from build123d import *

# Parameters (mm, degrees)
EXTRUDE_1_DEPTH      = 20
EXTRUDE_1_DEPTH_BACK = 10
SKETCH_1_R           = 11.4
SKETCH_2_R           = 12.5
EXTRUDE_2_DEPTH      = 30


with BuildPart() as part:
    # 草图1 → 凸台-拉伸1 (new, two sides: drawn at the far end of the back side and taken through both)
    with BuildSketch(Plane.XY.offset(-EXTRUDE_1_DEPTH_BACK)):
        Circle(SKETCH_1_R)
    extrude(amount=EXTRUDE_1_DEPTH + EXTRUDE_1_DEPTH_BACK)

    # 草图2 → 凸台-拉伸2 (add)
    with BuildSketch(Plane.XY.offset(20)):
        Circle(SKETCH_2_R)
    extrude(amount=EXTRUDE_2_DEPTH)

    # 草图7 → 切除-旋转1 (revolve, cut)
    with BuildSketch(Plane(origin=(0, 0, 0), x_dir=(0, 0, -1), z_dir=(1, 0, 0)), mode=Mode.PRIVATE) as cut_revolve_1_sk:
        Polygon((-50, 0), (-18, 0), (-22.506454643, 7.5), (-50, 7.5), align=None)
    revolve(cut_revolve_1_sk.sketch.rotate(Axis((0, 0, 50), (0, 0, -1)), 90), axis=Axis((0, 0, 50), (0, 0, -1)), mode=Mode.SUBTRACT)


solid = part.part
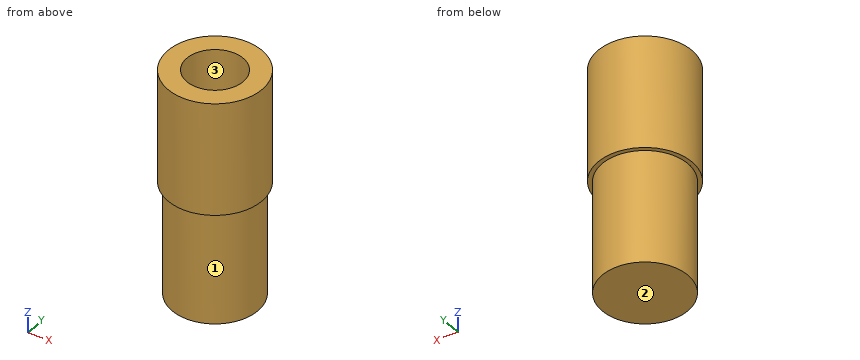
Build history of the part. All positions in model axes, mm. Face numbers are marked on the shaded views. Coordinates: 2 decimals unless noted, no trailing zeros. Order: outer loops, then holes, each group sorted by start corner. A loop starts at its lowest first (then second) coordinate and runs counter-clockwise, first axis right, second up. Notation, with made-up numbers: M 39.5,79 L 64.5,79 A7 cw 64.5,86 Z; hole C 38.5,32 d6. An arc over 180 degrees is marked long. One line per question, with ' | ' between items. Start each with the question number.
Q1. Saw through at A-A (x = -10.25). List the corners of the cut face in (y, z), then the cut area to 3 significant figures.
Q2. Saw through at D-D (y = 9). List the corners of the cut face in (x, z), then the cut area to 3 significant figures.
Q3. Saw through at C-C (z = 0.5). List the corners of the cut face in (x, y), then the cut area to 3 significant figures.
Q4. Flat gauge pins, fed straight in: pin 1 Ø6 at (x, z) = (-5, 28.5) entering from +Y; pin 2 Ø1.5 at (x, z) = (-6.5, 42) entering from +Y; pin 3 Ø4 at (y, z) = (-9, 17) entering from +X; pin 4 Ø1 at (x, y) = (9.5, -10) entering from -Z. Where does each tip first touch, or does it go through?
Q5. Saw through at B-B (z = 46.5). List the corners of the cut face in (x, y).
Q6. Two-plate mould, pull along X, no slides. Class the marked faces 1, 2 and 3: +X half, -X half, draft (parallel to the pull), parting line (faces both ways), or undercut.
Q7. Probe L1, parallel to Y at x = 0, z = 38.25; L2, parallel to X at y = -4, z = 47; L3, parallel to Y at x = -3.25, z = 42.5. List the from-to ranges inside material, lowest first. Write a range as from..to.
Check values:
1) outline: M -7.15,20 L -4.99,20 L -4.99,-10 L 4.99,-10 L 4.99,20 L 7.15,20 L 7.15,50 L -7.15,50 Z | area: 729 mm2
2) outline: M -8.67,20 L -7,20 L -7,-10 L 7,-10 L 7,20 L 8.67,20 L 8.67,50 L -8.67,50 Z | area: 940 mm2
3) outline: C 0,0 d22.8 | area: 408 mm2
4) pin 1: stops at y = 12.34 | pin 2: stops at y = 11.1 | pin 3: stops at x = 9 | pin 4: passes through
5) outline: C 0,0 d25; hole C 0,0 d15
6) face 1: parting line | face 2: draft | face 3: undercut
7) L1: y = -12.5..-7.5, 7.5..12.5 | L2: x = -11.84..-6.34, 6.34..11.84 | L3: y = -12.07..-6.76, 6.76..12.07
